from build123d import *

# Parameters (mm, degrees)
M12_TAPPED_HOLE1_D           = 10.2
M12_TAPPED_HOLE1_DEPTH       = 23.25
M12_TAPPED_HOLE1_CSINK_D     = 12.05
M12_TAPPED_HOLE1_CSINK_ANGLE = 90
M12_TAPPED_HOLE1_TIP         = 3.064389157
SKETCH4_R                    = 21.574990141
CUT_EXTRUDE1_DEPTH           = 15
CHAMFER1_SIZE                = 1.5


with BuildPart() as part:
    # Sketch1 → Revolve1 (revolve)
    with BuildSketch(Plane.XY, mode=Mode.PRIVATE) as revolve1_sk:
        Polygon((0, 0), (0, 10), (0.866025404, 11.5), (30, 11.5), (30, 6.5), (40, 6.5), (40, 11.5), (44, 11.5), (44, 5.5), (49, 5.5), (49, 8), (110, 8), (110, 0), align=None)
    revolve(revolve1_sk.sketch.rotate(Axis((0, 0, 0), (1, 0, 0)), 90), axis=Axis((0, 0, 0), (1, 0, 0)))

    # M12 Tapped Hole1
    with Locations(Plane(origin=(0, 0, 0), x_dir=(0, 0, -1), z_dir=(-1, 0, 0))):
        with Locations((0, 0)):
            CounterSinkHole(M12_TAPPED_HOLE1_D / 2, M12_TAPPED_HOLE1_CSINK_D / 2, depth=M12_TAPPED_HOLE1_DEPTH, counter_sink_angle=M12_TAPPED_HOLE1_CSINK_ANGLE)
            with Locations((0, 0, -(M12_TAPPED_HOLE1_DEPTH + M12_TAPPED_HOLE1_TIP / 2))):  # 118° drill point
                Cone(0, M12_TAPPED_HOLE1_D / 2, M12_TAPPED_HOLE1_TIP, mode=Mode.SUBTRACT)

    # Sketch4 → Cut-Extrude1 (cut)
    with BuildSketch(Plane.ZY):
        Circle(SKETCH4_R)
        Polygon((5.227352222, 10.296024576), (-6.30294273, 9.675032107), (-11.530294952, -0.620992469), (-5.227352222, -10.296024576), (6.30294273, -9.675032107), (11.530294952, 0.620992469), align=None, mode=Mode.SUBTRACT)
    extrude(amount=-CUT_EXTRUDE1_DEPTH, mode=Mode.SUBTRACT)

    # Chamfer1
    chamfer1_edges = [part.edges().sort_by_distance(p)[0] for p in [
        (110, 0, -8),
    ]]
    chamfer(chamfer1_edges, length=CHAMFER1_SIZE)


solid = part.part
The model under review builds one solid part; all positions refer to its coordinate system, in mm. A direction names the side the tool comes from. Round coordinates to 2 decimals unless told otherwise and drop trailing zeros. Loops run counter-clockwise (first coordinate to the right, second up) from the corner with the lowest first, then second, coordinate; pieces in that order, holes last. Notation, with made-up numbers: M 9.5,-17.75 L 47.5,-17.75 A31 cw 47.5,13.25 Z; hole C -6.75,-31 d9. An arc over 180 degrees is marked long. Answer as a JSON object with one key per item and string values.
Item 1: The part is to be moulded in two halves that separate along Y. For faces 1 (the face through (15, -6, -9)), 2 (the face through (12.2, 4.5, 2.4)), 3 (the face through (79.17, 7.81, -1.73)), say which applies: +Y half, -Y half, draft (parallel to the pull), parting line (faces both ways), or undercut.
Check sheet entries:
{"face 1": "draft", "face 2": "undercut", "face 3": "parting line"}
Item 2: We need section B-B, the plane x = 71. State the section outline as (y, z) points.
Check sheet entries:
{"outline": "C 0,0 d16"}
Item 3: For line 1 along X through (y, z) = (-5.75, 2); line 2 along Y through (x, z) = (8.5, 0); line 3 along X through (y, z) = (8.25, 0.5), list the stretches that pass through material, from the lowest coordinate up.
Check sheet entries:
{"line 1": "0 to 44, 49 to 110", "line 2": "-10.01 to -5.1, 5.1 to 10.01", "line 3": "0 to 30, 40 to 44"}
Item 4: We need section C-C, the plane x = 46. State the section outline as (y, z) points, and give its area (3 significant figures).
Check sheet entries:
{"outline": "C 0,0 d11", "area": "95.0 mm2"}
Item 5: Tool access review of faces 4 (the face through (7.39, -9.99, 0.46)), 5 (the face through (15, 5, -10)), 6 (the face through (35.07, 3.955, -5.158)): name each direction out of +Z, -Z, +X, -X, +Y, -Y from which nothing blocks a thin tool from reaching the whole face with its end or side.
Check sheet entries:
{"face 4": "+Z, -X, -Y", "face 5": "-Z, -X, +Y", "face 6": "none"}
Item 6: We need section A-A, the plane x = 10.5. State the section outline as (y, z) points, and give its area (3 significant figures).
Check sheet entries:
{"outline": "M -10.29,-5.13 A11.5 ccw -10.22,-5.28 L -0.7,-11.48 A11.5 ccw -0.54,-11.49 L 9.59,-6.35 A11.5 ccw 9.68,-6.21 L 10.29,5.13 A11.5 ccw 10.22,5.28 L 0.7,11.48 A11.5 ccw 0.54,11.49 L -9.59,6.35 A11.5 ccw -9.68,6.21 Z; hole C 0,0 d10.2", "area": "265 mm2"}
Item 7: Clearance check with flat-ended pins moving along their axes: P1, Ø1.5, axis at x = 22.5, z = -1, coming from the +Y side; P2, Ø1.5, axis at y = 2.5, z = -10, coming from the -X side; P3, Ø3, axis at x = 23.5, z = -6.5, coming from the -Y side; P4, Ø3, axis at y = 6.5, z = -7.5, coming from the +X side. State where each tip first meets the part, or that it passes through.
Check sheet entries:
{"P1": "y = 11.5", "P2": "x = 0", "P3": "y = -10.36", "P4": "x = 44"}
